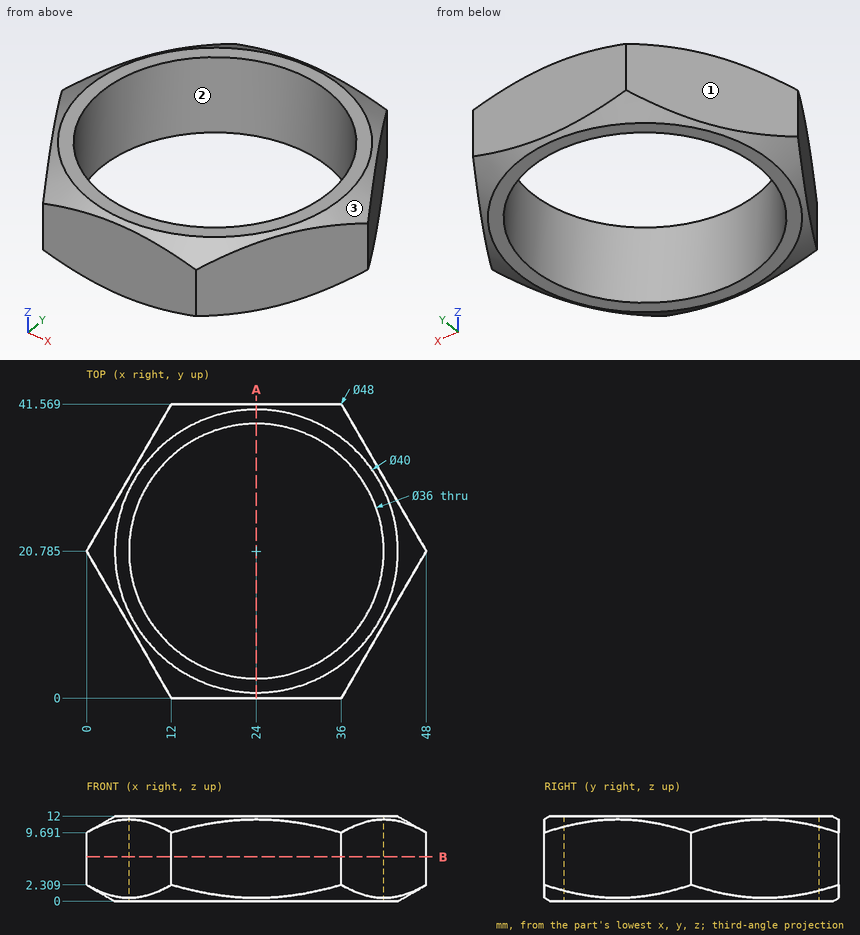
Geometry: see drawing. Coordinates: mm, zero at the bounding-box minimum. Give positions to 0.01 mm unless a question says otherwise; leave off trailing zeros. Write each loop counter-clockwise with the first axis right and the second up, starting at its lowest first coordinate (ties: lowest second). Pieces come first, ordered by that corner, then holes. Notation, with made-up numbers: (21, 40.5) - (39, 40.5) arc R30 ccw to (39, 72.5) - close; hole circle Ø7 at (30.25, 38.25). An arc over 180 degrees is marked (long way). Return JSON: item names as keys, results as strings. Group by question number.
1) Line query: line 1 (Y direction, x = 24, z = 9) (1 decimal); line 2 (X direction, y = 22, z = 2.75); line 3 (X direction, y = 28, z = 2) (1 decimal). Output: solid intervals per line, ascending.
2) First-contact query: P1, Ø5, axis at x = 5, z = 10.5, coming from the -Y side (1 decimal); P2, Ø5, axis at x = 6, z = 9, coming from the -Y side. Flat tips, straight axial feed; report the tip coordinate or a pass-through.
3) Section A-A on x = 24. Return the cut outline in (y, z) (1 decimal).
4) Mould query, pull axis Y, two halves, no side actions, for the marked faces 1, 2 and 3. Classes: released by +Y, released by -Y, zero draft, split by the parting line, or undercut.
5) Section B-B on z = 6.25. Return the cut outline in (x, y) (1 decimal).
Filled in:
{
 "1": {"line 1": "y = 0 to 2.8, 38.8 to 41.6", "line 2": "x = 0.7 to 6.04, 41.96 to 47.3", "line 3": "x = 4.2 to 7.5, 40.5 to 43.8"},
 "2": {"P1": "stops at y = 7.8", "P2": "stops at y = 6.06"},
 "3": {"outline": "(0, 0.5) - (0.8, 0) - (2.8, 0) - (2.8, 12) - (0.8, 12) - (0, 11.5) - close; (38.8, 0) - (40.8, 0) - (41.6, 0.5) - (41.6, 11.5) - (40.8, 12) - (38.8, 12) - close"},
 "4": {"face 1": "released by +Y", "face 2": "undercut", "face 3": "split by the parting line"},
 "5": {"outline": "(0, 20.8) - (12, 0) - (36, 0) - (48, 20.8) - (36, 41.6) - (12, 41.6) - close; hole circle Ø36 at (24, 20.8)"}
}
